For this review, take the finished solid that the model builds, in its own axes (mm). Give positions to 0.01 mm unless a question says otherwise; leave off trailing zeros. Write each loop counter-clockwise with the first axis right and the second up, starting at its lowest first coordinate (ties: lowest second). Pieces come first, ordered by that corner, then holes.
1) Wall thickness on line 1 along X through (y, z) = (1.75, 0); line 2 along Y through (x, z) = (-3, 3); line 3 along Z through (x, y) = (-0.25, 0.9): over which ranges is each line inside the solid? List them lowest first.
2) We need section A-A on x = 0. Give the boundary of the cut face in (y, z).
3) For P1, Ø3, axis at x = 0, z = 0, coming from the -Y side; P2, Ø2, axis at x = 0.5, y = 4.5, coming from the -Z side, all flat-tipped, find the tip position at first contact; note any pin that passes through.
4) We need section B-B on z = 0. Give the boundary of the cut face in (x, y).
5) We need section C-C on y = 4.2. Give the boundary of the cut face in (x, z).
6) Draft analysis for pull direction X (two halves, no side actions). For faces 1 (the face through (3.04, 0.25, 3.97)), 2 (the face through (2, 0, 2)), 3 (the face through (-0.1, 3, 2.5)), state which applies: pulls with the +X half, pulls with the -X half, needs draft (parallel to the pull), parting line crosses it, or undercut.
from build123d import *

# Parameters (mm, degrees)
CHAMFER_1_SIZE = 0.1


with BuildPart() as part:
    # 草图1 → 旋转1 (revolve)
    with BuildSketch(Plane.XY, mode=Mode.PRIVATE) as revolve_1_sk:
        Polygon((2.5, 0), (5, 0), (5, 0.5), (3, 0.5), (3, 6), (2.5, 6), align=None)
    revolve(revolve_1_sk.sketch.rotate(Axis((0, 0, 0), (0, 1, 0)), 90), axis=Axis((0, 0, 0), (0, 1, 0)))

    # 倒角1
    chamfer_1_edges = [part.edges().sort_by_distance(p)[0] for p in [
        (0, 6, 2.5),
        (0, 6, 3),
        (0, 0.5, 3),
        (0, 0.5, 5),
        (0, 0, 5),
        (0, 0, 2.5),
    ]]
    chamfer(chamfer_1_edges, length=CHAMFER_1_SIZE)


solid = part.part
Results list:
1. line 1: x = -3 to -2.5, 2.5 to 3
1. line 2: y = 0 to 0.5
1. line 3: z = -2.99 to -2.49, 2.49 to 2.99
2. outline: (0, -4.9) - (0.1, -5) - (0.4, -5) - (0.5, -4.9) - (0.5, -3.1) - (0.6, -3) - (5.9, -3) - (6, -2.9) - (6, -2.6) - (5.9, -2.5) - (0.1, -2.5) - (0, -2.6) - close; (0, 2.6) - (0.1, 2.5) - (5.9, 2.5) - (6, 2.6) - (6, 2.9) - (5.9, 3) - (0.6, 3) - (0.5, 3.1) - (0.5, 4.9) - (0.4, 5) - (0.1, 5) - (0, 4.9) - close
3. P1: passes through
3. P2: stops at z = -3
4. outline: (-5, 0.1) - (-4.9, 0) - (-2.6, 0) - (-2.5, 0.1) - (-2.5, 5.9) - (-2.6, 6) - (-2.9, 6) - (-3, 5.9) - (-3, 0.6) - (-3.1, 0.5) - (-4.9, 0.5) - (-5, 0.4) - close; (2.5, 0.1) - (2.6, 0) - (4.9, 0) - (5, 0.1) - (5, 0.4) - (4.9, 0.5) - (3.1, 0.5) - (3, 0.6) - (3, 5.9) - (2.9, 6) - (2.6, 6) - (2.5, 5.9) - close
5. outline: circle Ø6 at (0, 0); hole circle Ø5 at (0, 0)
6. face 1: parting line crosses it
6. face 2: needs draft
6. face 3: undercut
